Could you check a few things on this model? Use its own coordinates, in mm. A direction names the side the tool comes from. Give positions to 0.01 mm unless a question says otherwise; leave off trailing zeros. Loops run counter-clockwise (first coordinate to the right, second up) from the corner with the lowest first, then second, coordinate; pieces in that order, holes last. Notation, with made-up numbers: (39, 19.25) - (86, 19.25) arc R26 ccw to (86, 58.25) - close; hole circle Ø4 at (-19, 9.25). An arc over 180 degrees is marked (long way). Use CSV: the item, a comma, the result in double quotes.
from build123d import *

# Parameters (mm, degrees)
SKETCH1_W                                            = 8
SKETCH1_H                                            = 20
BOSS_EXTRUDE1_DEPTH                                  = 7.25
SKETCH2_W                                            = 5
SKETCH2_H                                            = 11.9
CUT_EXTRUDE1_DEPTH                                   = 9.1
CBORE_FOR_M2_5_HEX_SOCKET_HEAD_CAP_SCREW_D           = 2.9
CBORE_FOR_M2_5_HEX_SOCKET_HEAD_CAP_SCREW_CBORE_D     = 5.3
CBORE_FOR_M2_5_HEX_SOCKET_HEAD_CAP_SCREW_CBORE_DEPTH = 2.9
SKETCH7_W                                            = 11.4
SKETCH7_H                                            = 6.5
CUT_EXTRUDE3_DEPTH                                   = 15.716062653
CHAMFER1_SIZE                                        = 1
CHAMFER2_SIZE                                        = 5
CUT_EXTRUDE4_DEPTH                                   = 9.1


with BuildPart() as part:
    # Sketch1 → Boss-Extrude1 (new, symmetric)
    with BuildSketch(Plane(origin=(0, 0, 0), x_dir=(1, 0, 0), z_dir=(0, 1, 0))):
        Rectangle(SKETCH1_W, SKETCH1_H)
    extrude(amount=BOSS_EXTRUDE1_DEPTH, both=True)

    # Sketch2 → Cut-Extrude1 (cut)
    with BuildSketch(Plane.XZ.offset(7.25)):
        with Locations((0, 4.05)):
            Rectangle(SKETCH2_W, SKETCH2_H)
    extrude(amount=-CUT_EXTRUDE1_DEPTH, mode=Mode.SUBTRACT)

    # CBORE for M2.5 Hex Socket Head Cap Screw2 (through all)
    with Locations(Plane(origin=(0, 7.25, 0), x_dir=(1, 0, 0), z_dir=(0, 1, 0))):
        with Locations((0, -6.8), (0, -1.1)):
            CounterBoreHole(CBORE_FOR_M2_5_HEX_SOCKET_HEAD_CAP_SCREW_D / 2, CBORE_FOR_M2_5_HEX_SOCKET_HEAD_CAP_SCREW_CBORE_D / 2, CBORE_FOR_M2_5_HEX_SOCKET_HEAD_CAP_SCREW_CBORE_DEPTH)

    # Sketch7 → Cut-Extrude3 (cut, through all)
    with BuildSketch(Plane(origin=(4, 0, 0), x_dir=(0, 0, -1), z_dir=(1, 0, 0))):
        with Locations((-4.3, -4)):
            Rectangle(SKETCH7_W, SKETCH7_H)
    extrude(amount=-CUT_EXTRUDE3_DEPTH, mode=Mode.SUBTRACT)

    # Chamfer1
    chamfer1_edges = [part.edges().sort_by_distance(p)[0] for p in [
        (4, 3.25, 10),
        (-4, 3.25, 10),
    ]]
    chamfer(chamfer1_edges, length=CHAMFER1_SIZE)

    # Chamfer2
    chamfer2_edges = [part.edges().sort_by_distance(p)[0] for p in [
        (0, 7.25, -10),
    ]]
    chamfer(chamfer2_edges, length=CHAMFER2_SIZE)

    # Sketch6 → Cut-Extrude4 (cut)
    with BuildSketch(Plane.XZ.offset(7.25)):
        with BuildLine():
            Line((-4, 0.1), (4, 0.1))
            ThreePointArc((4, 0.1), (5, -0.9), (4, -1.9))
            Line((4, -1.9), (-4, -1.9))
            ThreePointArc((-4, -1.9), (-5, -0.9), (-4, 0.1))
        make_face()
    extrude(amount=-CUT_EXTRUDE4_DEPTH, mode=Mode.SUBTRACT)


solid = part.part
1) Suppose I cut it at A-A (z = 1.1). Please give me the cut outline in (x, y).
Answer below:
outline,"(-4, -0.75) - (-2.5, -0.75) - (-2.5, 1.85) - (-1.45, 1.85) - (-1.45, 4.35) - (-2.65, 4.35) - (-2.65, 7.25) - (-4, 7.25) - close; (1.45, 1.85) - (2.5, 1.85) - (2.5, -0.75) - (4, -0.75) - (4, 7.25) - (2.65, 7.25) - (2.65, 4.35) - (1.45, 4.35) - close"
2) Suppose I cut it at B-B (y = 0). Please give me the cut outline in (x, z), plus the area to 3 significant figures.
Answer below:
outline,"(-4, -10) - (4, -10) - (4, -1.9) - (-4, -1.9) - close; (-4, 0.1) - (-2.5, 0.1) - (-2.5, 10) - (-3, 10) - (-4, 9) - close; (2.5, 0.1) - (4, 0.1) - (4, 9) - (3, 10) - (2.5, 10) - close"
area,"93.5 mm2"
3) I'm going to push flat-ended pins straight in: P1, Ø1.6, axis at x = 3, z = 3, coming from the -Y side; P2, Ø1.6, axis at x = -1, z = 1, coming from the +Y side; P3, Ø4, axis at x = -1, y = 3, coming from the -Z side; P4, Ø4.5, axis at x = 0, z = 1.1, coming from the -Y side. Where does each tip first touch, or does it pass through?
Answer below:
P1,"stops at y = -0.75"
P2,"stops at y = 4.35"
P3,"stops at z = -10"
P4,"stops at y = 1.85"
4) Which directions (+Z, -Z, +X, -X, +Y, -Y) give clear straight access to the entire face, cutting with the end or side of a thin tool? Please do faces 1 (the flat face through (-2.5, 1, 5)), 2 (the cylindrical face through (0.314, 3.082, 8.216)), 3 (the flat face through (3, 1, 0.1)), 4 (the flat face through (-3, -0.75, 5)), 5 (the flat face through (1.14, 4.35, 2.24)).
Answer below:
face 1,"+Z, -Y"
face 2,"+Y, -Y"
face 3,"+X, -X, -Y"
face 4,"+Z, +X, -X, -Y"
face 5,"+Y"
5) Suppose I cut it at D-D (x = -2.25). Please give me the cut outline in (y, z).
Answer below:
outline,"(-7.25, -10) - (2.25, -10) - (7.25, -5) - (7.25, -0.3) - (4.35, -0.3) - (4.35, 2.5) - (7.25, 2.5) - (7.25, 5.4) - (4.35, 5.4) - (4.35, 8.2) - (7.25, 8.2) - (7.25, 10) - (1.85, 10) - (1.85, -1.9) - (-7.25, -1.9) - close"
6) Suppose I cut it at C-C (x = 0). Please give me the cut outline in (y, z), plus the area to 3 significant figures.
Answer below:
outline,"(-7.25, -10) - (2.25, -10) - (7.25, -5) - (7.25, -1.55) - (4.35, -1.55) - (4.35, -0.35) - (1.85, -0.35) - (1.85, -1.9) - (-7.25, -1.9) - close; (1.85, 2.55) - (4.35, 2.55) - (4.35, 3.75) - (7.25, 3.75) - (7.25, 4.15) - (4.35, 4.15) - (4.35, 5.35) - (1.85, 5.35) - close; (1.85, 8.25) - (4.35, 8.25) - (4.35, 9.45) - (7.25, 9.45) - (7.25, 10) - (1.85, 10) - close"
area,"124 mm2"
7) I need wall thicknesses on line 1 along Z through (x, y) = (0.75, 4.5); line 2 along X through (y, z) = (1.5, 7); line 3 along Z through (x, y) = (0, 3.55). Which ranges of each line are inside material? Lowest first, please.
Answer below:
line 1,"z = -7.75 to -1.44, 3.64 to 4.26, 9.34 to 10"
line 2,"x = -4 to -2.5, 2.5 to 4"
line 3,"z = -8.7 to -0.35, 2.55 to 5.35, 8.25 to 10"
